Geometry: final body of the model. Coordinates: model frame, mm. A direction names the side the tool comes from. Give positions to 0.01 mm unless a question says otherwise; leave off trailing zeros. Write each loop counter-clockwise with the first axis right and the second up, starting at its lowest first coordinate (ties: lowest second). Pieces come first, ordered by that corner, then holes. Notation, with made-up numbers: M -30.5,-19.75 L -22.5,-19.75 A25 cw -22.5,6.25 Z; hole C 17.5,59 d4. An arc over 180 degrees is marked long. One line per question, with ' | ' between items.
from build123d import *

# Parameters (mm, degrees)
SKETCH1_R             = 3
BOSS_EXTRUDE1_DEPTH   = 8
CHAMFER1_SIZE         = 0.5
M3_TAPPED_HOLE1_D     = 2.5
M3_TAPPED_HOLE1_DEPTH = 6.5
M3_TAPPED_HOLE1_TIP   = 0.751075774
SKETCH3_W             = 0.3
SKETCH3_H             = 0.2


with BuildPart() as part:
    # Sketch1 → Boss-Extrude1 (new body)
    with BuildSketch(Plane(origin=(0, 0, 0), x_dir=(0, 0, -1), z_dir=(1, 0, 0))):
        Circle(SKETCH1_R)
    extrude(amount=BOSS_EXTRUDE1_DEPTH)

    # Chamfer1
    chamfer1_edges = [part.edges().sort_by_distance(p)[0] for p in [
        (8, 0, 3),
    ]]
    chamfer(chamfer1_edges, length=CHAMFER1_SIZE)

    # M3 Tapped Hole1
    with Locations(Plane(origin=(0, 0, 0), x_dir=(0, 0, -1), z_dir=(-1, 0, 0))):
        with Locations((0, 0)):
            Hole(M3_TAPPED_HOLE1_D / 2, depth=M3_TAPPED_HOLE1_DEPTH)
            with Locations((0, 0, -(M3_TAPPED_HOLE1_DEPTH + M3_TAPPED_HOLE1_TIP / 2))):  # 118° drill point
                Cone(0, M3_TAPPED_HOLE1_D / 2, M3_TAPPED_HOLE1_TIP, mode=Mode.SUBTRACT)

    # Sketch3 → Cut-Revolve1 (revolve, cut)
    with BuildSketch(Plane(origin=(0, 0, 0), x_dir=(1, 0, 0), z_dir=(0, 1, 0)), mode=Mode.PRIVATE) as cut_revolve1_sk:
        with Locations((6.25, 2.9)):
            Rectangle(SKETCH3_W, SKETCH3_H)
    revolve(cut_revolve1_sk.sketch.rotate(Axis((0, 0, 0), (1, 0, 0)), 180), axis=Axis((0, 0, 0), (1, 0, 0)), mode=Mode.SUBTRACT)


solid = part.part
(1) Cut plane B-B, the plane x = 7. Return loops of the section in (y, z).
Working result:
outline: C 0,0 d6; hole C 0,0 d0.84
(2) Set-up query: faces 4 (the face through (6.25, -0.84, 2.67)), 5 (the face through (0, -1, -1)). Return all of +Z, -Z, +X, -X, +Y, -Y with unobstructed straight access to the full face (end or side cutting, diameter ignored); none if empty.
Working result:
face 4: none | face 5: +Z, -Z, -X, +Y, -Y
(3) First-contact query: P1, Ø1.5, axis at x = 2, z = -1.5, coming from the +Y side; P2, Ø1.5, axis at y = 0, z = 0, coming from the -X side; P3, Ø1.5, axis at x = 4, y = -2, coming from the +Z side. Flat tips, straight axial feed; report the tip coordinate or a pass-through.
Working result:
P1: stops at y = 2.9 | P2: stops at x = 6.8 | P3: stops at z = 2.73
(4) Cut plane A-A, the plane x = 6. Return loops of the section in (y, z).
Working result:
outline: C 0,0 d6; hole C 0,0 d2.5
(5) Material intervals for L1, parallel to Y at x = 3.75, z = 0; L2, parallel to X at y = 1.8, z = -2.2; L3, parallel to Z at x = 3.25, y = -1.1, sorted ascending. Write a range as [from, to].
Working result:
L1: y = [-3, -1.25], [1.25, 3] | L2: x = [0, 6.1], [6.4, 7.66] | L3: z = [-2.79, -0.59], [0.59, 2.79]
(6) Draft query along Z for faces 1 (the face through (3, 0, 3)), 2 (the face through (8, 0, 0)), 3 (the face through (3.3, 1.22, -0.27)). Return one class per face: released by +Z, released by -Z, zero draft, split by the parting line, or undercut.
Working result:
face 1: split by the parting line | face 2: zero draft | face 3: undercut
